from build123d import *

# Parameters (mm, degrees)
FORK_BODY_DEPTH         = 200
SIDE_BOSS_A_SKETCH_R    = 40
SIDE_BOSS_A_DEPTH       = 40
SIDE_START              = 40
SIDE_BOSS_B_SKETCH_R    = 40
SIDE_BOSS_B_DEPTH       = 40
PIVOT_BORE_SKETCH_R     = 40
PIVOT_BORE_80_DEPTH     = 516.460958754
TOP_LUG_SKETCH_R        = 40
TOP_LUG_DEPTH           = 25
TOP_LUG_BLEND_R20_R     = 20
FORK_FILLET_R40_A_R     = 40
FORK_FILLET_R40_B_R     = 40
FORK_FILLET_R40_C_R     = 40
FORK_FILLET_R40_D_R     = 40
FOOT_SLOTS_15X120_DEPTH = 536.253402042


with BuildPart() as part:
    # Fork Profile Sketch → Fork Body (new body)
    with BuildSketch(Plane.XY):
        Polygon((0, 0), (-100, 0), (-100, -200), (-139.993222056, -330), (-139.993222056, -410), (-99.993222056, -410), (-99.993222056, -330), (-60, -200), (-60, -40), (60, -40), (60, -200), (99.993222056, -330), (99.993222056, -410), (139.993222056, -410), (139.993222056, -330), (100, -200), (100, 0), align=None)
    extrude(amount=-FORK_BODY_DEPTH)

    # Side Boss A Sketch → Side Boss A (add)
    with BuildSketch(Plane(origin=(140, 0, 0), x_dir=(0, 0, -1), z_dir=(1, 0, 0))):
        with BuildLine():
            Line((75, -170.710678119), (75, -330))
            Line((75, -330), (125, -330))
            Line((125, -330), (125, -170.710678119))
            ThreePointArc((125, -170.710678119), (100, -25), (75, -170.710678119))
        make_face()
        with Locations((100, -100)):
            Circle(SIDE_BOSS_A_SKETCH_R, mode=Mode.SUBTRACT)
    extrude(amount=-SIDE_BOSS_A_DEPTH)

    # Side Boss B Sketch → Side Boss B (add)
    with BuildSketch(Plane(origin=(-140, 0, 0), x_dir=(0, 0, -1), z_dir=(1, 0, 0)).offset(SIDE_START)):
        with BuildLine():
            Line((125, -170.710678119), (125, -330))
            Line((125, -330), (75, -330))
            Line((75, -330), (75, -170.710678119))
            ThreePointArc((75, -170.710678119), (100, -25), (125, -170.710678119))
        make_face()
        with Locations((100, -100)):
            Circle(SIDE_BOSS_B_SKETCH_R, mode=Mode.SUBTRACT)
    extrude(amount=-SIDE_BOSS_B_DEPTH)

    # Pivot Bore Sketch → Pivot Bore Ø80 (cut, through all)
    with BuildSketch(Plane(origin=(100, 0, 0), x_dir=(0, 0, -1), z_dir=(1, 0, 0))):
        with Locations((100, -100)):
            Circle(PIVOT_BORE_SKETCH_R)
    extrude(amount=-PIVOT_BORE_80_DEPTH, mode=Mode.SUBTRACT)

    # Top Lug Sketch → Top Lug (add, symmetric)
    with BuildSketch(Plane.XY.offset(-100)):
        with BuildLine():
            Line((-100, 90), (-100, 0))
            Line((-100, 0), (100, 0))
            Line((100, 0), (100, 90))
            ThreePointArc((100, 90), (0, 190), (-100, 90))
        make_face()
        with Locations((0, 90)):
            Circle(TOP_LUG_SKETCH_R, mode=Mode.SUBTRACT)
    extrude(amount=TOP_LUG_DEPTH, both=True)

    # Top Lug Blend R20
    top_lug_blend_r20_edges = [part.edges().sort_by_distance(p)[0] for p in [
        (0, 0, -75),
        (0, 0, -125),
        (0, 0, 0),
        (0, 0, -200),
    ]]
    fillet(top_lug_blend_r20_edges, radius=TOP_LUG_BLEND_R20_R)

    # Fork Fillet R40 A
    fork_fillet_r40_a_edges = [part.edges().sort_by_distance(p)[0] for p in [
        (119.993222056, -410, 0),
    ]]
    fillet(fork_fillet_r40_a_edges, radius=FORK_FILLET_R40_A_R)

    # Fork Fillet R40 B
    fork_fillet_r40_b_edges = [part.edges().sort_by_distance(p)[0] for p in [
        (119.993222056, -410, -200),
    ]]
    fillet(fork_fillet_r40_b_edges, radius=FORK_FILLET_R40_B_R)

    # Fork Fillet R40 C
    fork_fillet_r40_c_edges = [part.edges().sort_by_distance(p)[0] for p in [
        (-119.993222056, -410, 0),
    ]]
    fillet(fork_fillet_r40_c_edges, radius=FORK_FILLET_R40_C_R)

    # Fork Fillet R40 D
    fork_fillet_r40_d_edges = [part.edges().sort_by_distance(p)[0] for p in [
        (-119.993222056, -410, -200),
    ]]
    fillet(fork_fillet_r40_d_edges, radius=FORK_FILLET_R40_D_R)

    # Foot Slot Sketch → Foot Slots 15x120 (cut, through all)
    with BuildSketch(Plane(origin=(139.993222056, 0, 0), x_dir=(0, 0, -1), z_dir=(1, 0, 0))):
        with BuildLine():
            Line((40, -355), (160, -355))
            ThreePointArc((160, -355), (175, -370), (160, -385))
            Line((160, -385), (40, -385))
            ThreePointArc((40, -385), (25, -370), (40, -355))
        make_face()
    extrude(amount=-FOOT_SLOTS_15X120_DEPTH, mode=Mode.SUBTRACT)


solid = part.part
Geometry check sheet. Reference: the model listing, model coordinates, mm. A direction names the side the tool comes from. Give positions to 0.01 mm unless a question says otherwise; leave off trailing zeros. Order: outer loops, then holes, each group sorted by start corner. A loop starts at its lowest first (then second) coordinate and runs counter-clockwise, first axis right, second up.
1. Sectioned sample at C-C (z = -100). State how many separate pieces and enclosed holes the cut face has, then the cut area to 3 significant figures.
Completed:
separate pieces: 5
enclosed holes: 1
area: 70,300 mm2
2. Scan lines: line 1 (Y direction, x = 108.5, z = -100); line 2 (Y direction, x = 0, z = -87); line 3 (X direction, y = -122, z = -36). Record each from-to range of solid material in increasing order.
Completed:
line 1: y = -410 to -385, -355 to -140, -60 to -25
line 2: y = -40 to 50, 130 to 190
line 3: x = -140 to -60, 60 to 140
3. Depth check by flat-ended pin: pin 1 (17.5 mm diameter, centred on x = 48.5, z = -154, fed in from +Y); pin 2 (24 mm diameter, centred on y = -385, z = -65.5, fed in from -X); pin 3 (6 mm diameter, centred on x = -92, y = 41, fed in from +Z). Enter the tip coordinate at first touch or a pass-through.
Completed:
pin 1: stops at y = 0
pin 2: stops at x = -139.99
pin 3: stops at z = -75
4. Sectioned sample at D-D (y = -336.5). Record the boundary of the cut face in (x, z), then the cut area to 3 significant figures.
Completed:
outline: (-139.99, -200) - (-99.99, -200) - (-99.99, 0) - (-139.99, 0) - close; (99.99, -200) - (139.99, -200) - (139.99, 0) - (99.99, 0) - close
area: 16,000 mm2
5. Sectioned sample at A-A (y = -100). Record the boundary of the cut face in (x, z), then the cut area to 3 significant figures.
Completed:
outline: (-140, -175) - (-100, -175) - (-100, -200) - (-60, -200) - (-60, -140) - (-140, -140) - close; (-140, -60) - (-60, -60) - (-60, 0) - (-100, 0) - (-100, -25) - (-140, -25) - close; (60, -200) - (100, -200) - (100, -175) - (140, -175) - (140, -140) - (60, -140) - close; (60, -60) - (140, -60) - (140, -25) - (100, -25) - (100, 0) - (60, 0) - close
area: 15,200 mm2
6. Draft check along Y on faces 6 (the face through (-120, -355, -99)), 7 (the face through (-140, -141, -101)), 8 (the face through (2.199, 189.976, -99.65)), 9 (the face through (-1, -40, -99)). Enter one of: pulls with the +Y half, pulls with the -Y half, needs draft (parallel to the pull), parting line crosses it, or undercut.
Completed:
face 6: undercut
face 7: needs draft
face 8: pulls with the +Y half
face 9: pulls with the -Y half
7. Access from +Z, -Z, +X, -X, +Y, -Y to the whole of each face (thin tool, end or side, straight path). Record for faces 1 (the face through (120, -385, -101)), 2 (the face through (125, -234, -125)), 3 (the face through (1, 0, -37)), 4 (the face through (120.277, -265.91, -36.975)), 5 (the face through (-119.72, -25.058, -97.059)).
Completed:
face 1: +X, -X
face 2: -Z, +X
face 3: +Z, +X, -X, +Y
face 4: +Z, +X
face 5: -X
8. Sectioned sample at B-B (x = 0). Record the boundary of the cut face in (y, z).
Completed:
outline: (-40, -200) - (-20, -200) arc R20 ccw to (0, -180) - (0, -145) arc R20 cw to (20, -125) - (50, -125) - (50, -75) - (20, -75) arc R20 cw to (0, -55) - (0, -20) arc R20 ccw to (-20, 0) - (-40, 0) - close; (130, -125) - (190, -125) - (190, -75) - (130, -75) - close
